Build history of the part. All positions in model axes, mm. Round coordinates to 2 decimals unless told otherwise and drop trailing zeros. Write each loop counter-clockwise with the first axis right and the second up, starting at its lowest first coordinate (ties: lowest second). Pieces come first, ordered by that corner, then holes. Notation, with made-up numbers: (-15.5, -23.75) -> (35.5, -23.75) arc R26 cw to (35.5, 1.25) -> close; hole circle Ø10 at (-21.5, -23.75). An arc over 180 degrees is marked (long way). Answer in a Markdown table with one row per item.
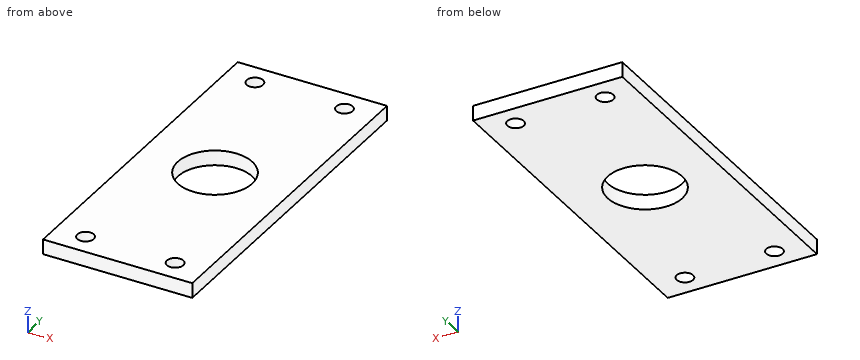
```python
from build123d import *

# Parameters (mm, degrees)
SKETCH_1_W          = 100
SKETCH_1_H          = 230
SKETCH_1_R          = 25
SKETCH_1_R_2        = 5.5
BOSS_EXTRUDE1_DEPTH = 10


with BuildPart() as part:
    # Sketch 1 → Boss-Extrude1 (new body)
    with BuildSketch(Plane.XY):
        Rectangle(SKETCH_1_W, SKETCH_1_H)
        Circle(SKETCH_1_R, mode=Mode.SUBTRACT)
        with Locations((-30, 100)):
            Circle(SKETCH_1_R_2, mode=Mode.SUBTRACT)
        with Locations((30, 100)):
            Circle(SKETCH_1_R_2, mode=Mode.SUBTRACT)
        with Locations((30, -100)):
            Circle(SKETCH_1_R_2, mode=Mode.SUBTRACT)
        with Locations((-30, -100)):
            Circle(SKETCH_1_R_2, mode=Mode.SUBTRACT)
    extrude(amount=BOSS_EXTRUDE1_DEPTH)


solid = part.part
```
Q1. Saw through at C-C on z = 6.25. Write the cut outline in (x, y).
A:
| item | result |
|---|---|
| outline | (-50, -115) -> (50, -115) -> (50, 115) -> (-50, 115) -> close; hole circle Ø11 at (-30, -100); hole circle Ø11 at (-30, 100); hole circle Ø50 at (0, 0); hole circle Ø11 at (30, -100); hole circle Ø11 at (30, 100) |
Q2. Drop flat-ended pins along their axis: P1, Ø12.5, axis at x = 30, y = 100, coming from the -Z side; P2, Ø1.5, axis at x = 5, y = -22, coming from the -Z side. Give the stop position or say it passes through.
A:
| item | result |
|---|---|
| P1 | z = 0 |
| P2 | through |
Q3. Saw through at D-D on y = 0. Write the cut outline in (x, z).
A:
| item | result |
|---|---|
| outline | (-50, 0) -> (-25, 0) -> (-25, 10) -> (-50, 10) -> close; (25, 0) -> (50, 0) -> (50, 10) -> (25, 10) -> close |
Q4. Saw through at B-B on x = 30. Write the cut outline in (y, z).
A:
| item | result |
|---|---|
| outline | (-115, 0) -> (-105.5, 0) -> (-105.5, 10) -> (-115, 10) -> close; (-94.5, 0) -> (94.5, 0) -> (94.5, 10) -> (-94.5, 10) -> close; (105.5, 0) -> (115, 0) -> (115, 10) -> (105.5, 10) -> close |
Q5. Wall check: line 1 (Y direction, x = 30, z = 7.5); line 2 (Y direction, x = 0, z = 4.25); line 3 (Y direction, x = -33, z = 1.5). Give the ranges that are in metal, low to high. Write a range as [from, to].
A:
| item | result |
|---|---|
| line 1 | [-115, -105.5], [-94.5, 94.5], [105.5, 115] |
| line 2 | [-115, -25], [25, 115] |
| line 3 | [-115, -104.61], [-95.39, 95.39], [104.61, 115] |
Q6. Saw through at A-A on y = 100. Write the cut outline in (x, z).
A:
| item | result |
|---|---|
| outline | (-50, 0) -> (-35.5, 0) -> (-35.5, 10) -> (-50, 10) -> close; (-24.5, 0) -> (24.5, 0) -> (24.5, 10) -> (-24.5, 10) -> close; (35.5, 0) -> (50, 0) -> (50, 10) -> (35.5, 10) -> close |
